Can you work these out from the drawing? Everything is in mm from the part's minimum corner. Coordinates: 2 decimals unless noted, no trailing zeros. Order: outer loops, then holes, each group sorted by start corner. A loop starts at its lowest first (then second) coordinate and runs counter-clockwise, first axis right, second up. Notation, with made-up numbers: (-22, 5) - (-14, 5) arc R13 ccw to (-14, 14) - close; hole circle Ø5 at (-27.5, 79). An arc over 180 degrees is marked (long way). Use a Markdown table: item, result. Add a question column.
(1) I want a section at B-B (y = 8.25). State how many separate pieces and enclosed holes the cut face has, and give its area (3 significant figures).
(2) I want a section at A-A (y = 15.5). List the corners of the cut face in (x, z) for me.
(3) I want a section at C-C (x = 92). List the corners of the cut face in (y, z) for me.
(4) For pin 1 Ø1.5 at (y, z) = (14, 69.5) entering from -X; pin 2 Ø7 at (x, z) = (75, 50) entering from +Y; pin 3 Ø4 at (x, y) = (43, 17.5) entering from -Z, each with a flat end and sliding along its axis, tell me the tip position at first contact or that it passes through.
(5) I want a section at D-D (z = 86). List the corners of the cut face in (x, y) for me.
(6) If I drill on L1, parallel to Z at x = 52, y = 14.25; L2, parallel to X at y = 5.5, z = 21.5; L3, parallel to Z at x = 100, y = 5, over which ranges is the centre line in solid material (lowest first)? Write a range as [from, to].
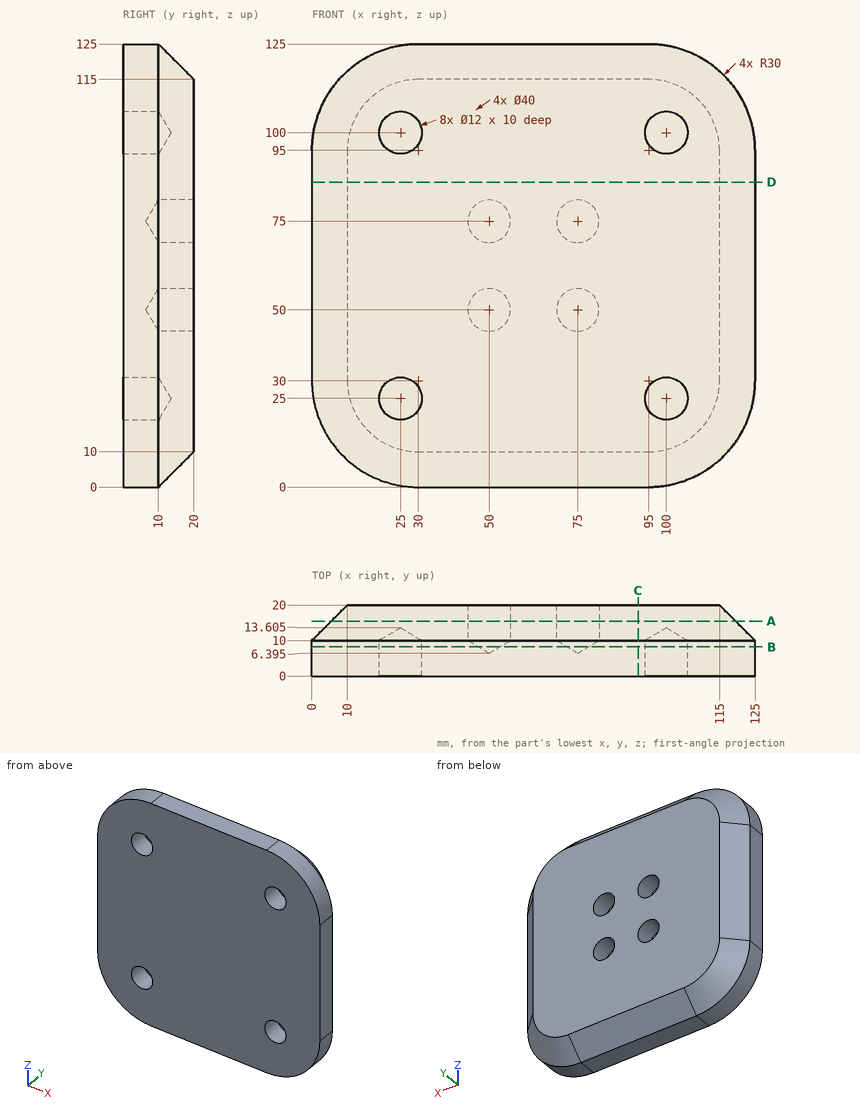
Answers follow:
| question | item | result |
|---|---|---|
| 1 | separate pieces | 1 |
| 1 | enclosed holes | 8 |
| 1 | area | 14,300 mm² |
| 2 | outline | (5.5, 30) arc R24.5 ccw to (30, 5.5) - (95, 5.5) arc R24.5 ccw to (119.5, 30) - (119.5, 95) arc R24.5 ccw to (95, 119.5) - (30, 119.5) arc R24.5 ccw to (5.5, 95) - close; hole circle Ø12 at (50, 50); hole circle Ø12 at (50, 75); hole circle Ø12 at (75, 50); hole circle Ø12 at (75, 75) |
| 3 | outline | (0, 0) - (10, 0) - (20, 10) - (20, 115) - (10, 125) - (0, 125) - close |
| 4 | pin 1 | stops at x = 3.25 |
| 4 | pin 2 | stops at y = 8.5 |
| 4 | pin 3 | stops at z = 5.5 |
| 5 | outline | (0, 0) - (125, 0) - (125, 10) - (115, 20) - (10, 20) - (0, 10) - close |
| 6 | L1 | z = [4.25, 44.34], [55.66, 69.34], [80.66, 120.75] |
| 6 | L2 | x = [1.23, 20.13], [29.87, 95.13], [104.87, 123.77] |
| 6 | L3 | z = [0.42, 19], [31, 94], [106, 124.58] |
